Check sheet for the drawn part. Datum: minimum x, y, z corner. Units: mm. A direction names the side the tool comes from. Give positions to 0.01 mm unless a question says otherwise; leave off trailing zeros. Write each loop counter-clockwise with the first axis right and the second up, starting at its lowest first coordinate (ties: lowest second). Pieces come first, ordered by that corner, then holes.
(1) Depth check by flat-ended pin: P1, Ø1.5, axis at x = 8, z = 57.5, coming from the -Y side; P2, Ø24, axis at y = 35, z = 20, coming from the +X side. Enter the tip coordinate at first touch or a pass-through.
(2) Cross-section at A-A (y = 35). Record the boundary of the cut face in (x, z), and give its area (3 significant figures).
(3) Cross-section at D-D (y = 56). Record the boundary of the cut face in (x, z), and give its area (3 significant figures).
(4) Cross-section at C-C (x = 19). Record the boundary of the cut face in (y, z).
(5) Tool access check on the marked faces 1 and 2. Record the directions out of +Z, -Z, +X, -X, +Y, -Y that give a thin tool (end or side, any length) a straight path to the whole face; none if there is none.
(6) Thickness scan on line 1 along Y through (x, z) = (24.5, 27); line 2 along X through (y, z) = (6, 36.5); line 3 along Y through (x, z) = (1, 20). Record the ranges inside material, lowest first.
(7) Cross-section at B-B (z = 20). Record the boundary of the cut face in (x, y), and give its area (3 significant figures).
(8) Mould release check, pull along Y, two halves, no side actions. Record for the marked faces 3, 4 and 5: +Y half, -Y half, draft (parallel to the pull), parting line (faces both ways), or undercut.
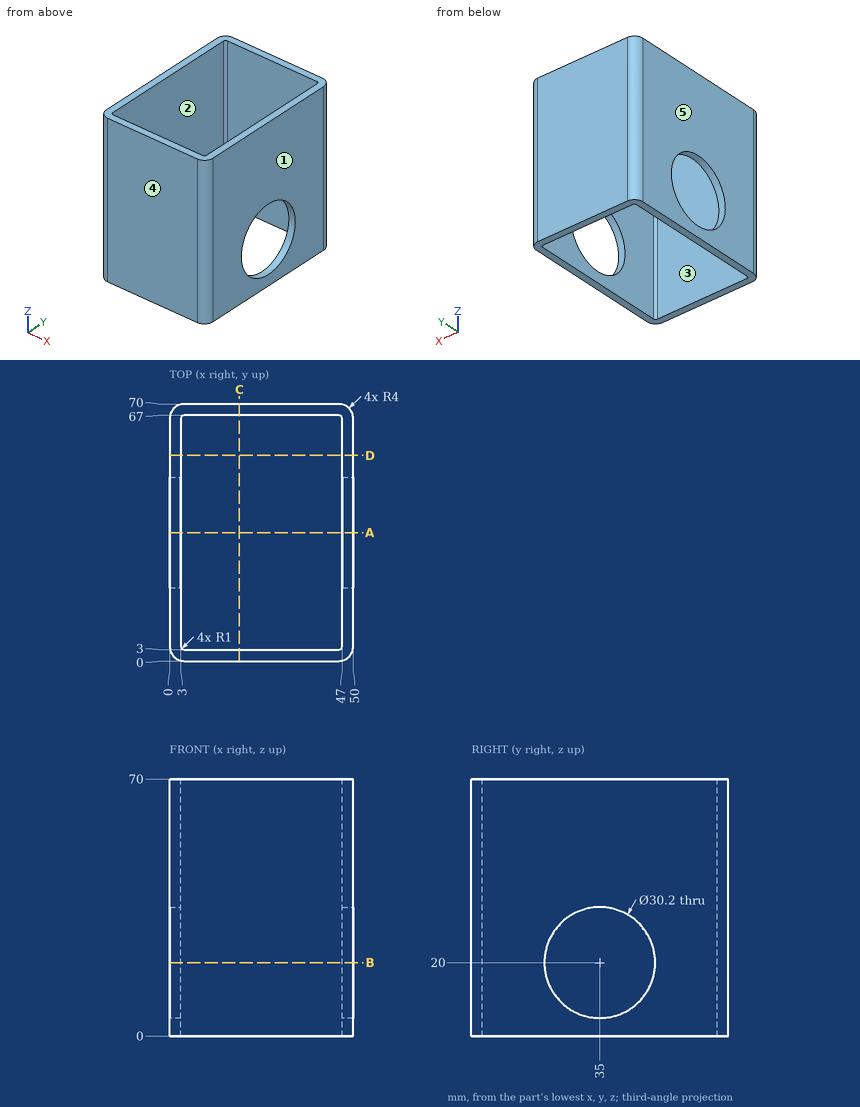
Reply:
1. P1: stops at y = 0
1. P2: passes through
2. outline: (0, 0) - (3, 0) - (3, 4.9) - (0, 4.9) - close; (0, 35.1) - (3, 35.1) - (3, 70) - (0, 70) - close; (47, 0) - (50, 0) - (50, 4.9) - (47, 4.9) - close; (47, 35.1) - (50, 35.1) - (50, 70) - (47, 70) - close
2. area: 239 mm2
3. outline: (0, 0) - (3, 0) - (3, 70) - (0, 70) - close; (47, 0) - (50, 0) - (50, 70) - (47, 70) - close
3. area: 420 mm2
4. outline: (0, 0) - (3, 0) - (3, 70) - (0, 70) - close; (67, 0) - (70, 0) - (70, 70) - (67, 70) - close
5. face 1: +Z, -Z, +X, +Y, -Y
5. face 2: +Z, -Z
6. line 1: y = 0 to 3, 67 to 70
6. line 2: x = 0 to 3, 47 to 50
6. line 3: y = 1.35 to 19.9, 50.1 to 68.65
7. outline: (0, 4) arc R4 ccw to (4, 0) - (46, 0) arc R4 ccw to (50, 4) - (50, 19.9) - (47, 19.9) - (47, 4) arc R1 cw to (46, 3) - (4, 3) arc R1 cw to (3, 4) - (3, 19.9) - (0, 19.9) - close; (0, 50.1) - (3, 50.1) - (3, 66) arc R1 cw to (4, 67) - (46, 67) arc R1 cw to (47, 66) - (47, 50.1) - (50, 50.1) - (50, 66) arc R4 ccw to (46, 70) - (4, 70) arc R4 ccw to (0, 66) - close
7. area: 490 mm2
8. face 3: undercut
8. face 4: -Y half
8. face 5: draft
